The model under review builds one solid part; all positions refer to its coordinate system, in mm. Coordinates: 2 decimals unless noted, no trailing zeros. Loops run counter-clockwise (first coordinate to the right, second up) from the corner with the lowest first, then second, coordinate; pieces in that order, holes last. Notation, with made-up numbers: (63.25, 70) - (79.25, 70) arc R17 ccw to (79.25, 90) - close; hole circle Ø4 at (51, 2.25). An arc over 180 degrees is marked (long way). Answer in a Markdown table with one row per item. Add a question column.
(1) For P1, Ø6, axis at y = -386.5, z = 2, coming from the -X side; P2, Ø3, axis at x = -726, z = 7.5, coming from the +Y side; P3, Ø4, axis at y = -235, z = 6.5, coming from the +X side, all flat-tipped, find the tip position at first contact; note any pin that passes through.
(2) We need section A-A on z = -6.75. Write out the cut boundary in (x, y).
(3) We need section C-C on y = -370. Write out the cut boundary in (x, z), plus the area to 3 significant figures.
(4) For line 1 along Y through (x, z) = (-836.5, -0.25); line 2 along Y through (x, z) = (-935, 2.75); line 3 along X through (y, z) = (-207.5, 0.75), list the stretches that pass through material, from the lowest coordinate up.
(5) We need section B-B on x = -821.5. Write out the cut boundary in (y, z).
from build123d import *

# Parameters (mm, degrees)
SKETCH2_W = 20
SKETCH2_H = 6


with BuildPart() as part:
    # Sweep1: sweep along a path in Sketch1
    with BuildLine(Plane.XY) as sweep1_path:
        Line((-803.471602915, -72.580053696), (-137.514764545, -198.618968438))
        ThreePointArc((-137.514764545, -198.618968438), (-117.217555143, -221.543328014), (-134.339730828, -246.927064367))
        Line((-134.339730828, -246.927064367), (-778.071333179, -459.044821132))
        ThreePointArc((-778.071333179, -459.044821132), (-1040.232770199, -282.208199453), (-803.471602915, -72.580053696))
    # Sketch2 → Sweep1 (sweep)
    with BuildSketch(Plane(origin=(-803.471602915, 0, 0), x_dir=(0, 0, -1), z_dir=(1, 0, 0))):
        with Locations((0, -75.580053696)):
            Rectangle(SKETCH2_W, SKETCH2_H)
    sweep(path=sweep1_path.line)


solid = part.part
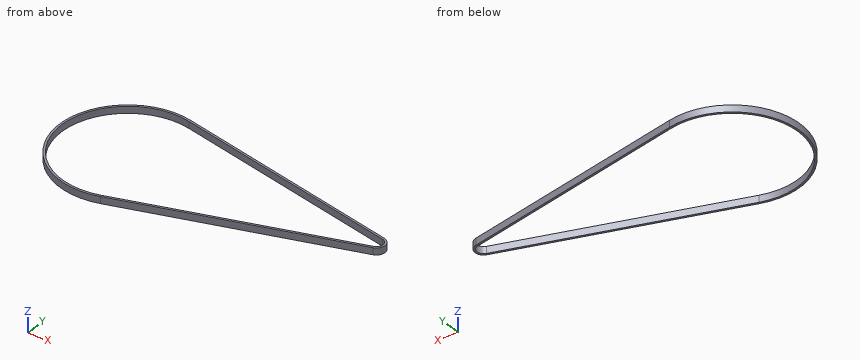
Outcome:
| question | item | result |
|---|---|---|
| 1 | P1 | x = -1004.71 |
| 1 | P2 | y = -86.96 |
| 1 | P3 | x = -119.17 |
| 2 | outline | (-803.47, -72.58) arc R200 ccw (long way) to (-778.07, -459.04) - (-134.34, -246.93) arc R25 ccw to (-137.51, -198.62) - close; hole (-803.47, -78.58) arc R194.11 ccw (long way) to (-780.98, -453.79) - (-137.24, -241.68) arc R19.14 ccw to (-137.51, -204.62) - close |
| 3 | outline | (-1013.34, -10) - (-1006.48, -10) - (-1006.48, 10) - (-1013.34, 10) - close; (-526.68, -10) - (-507.84, -10) - (-507.84, 10) - (-526.68, 10) - close |
| 3 | area | 514 mm² |
| 4 | line 1 | -469.05 to -463.15, -75.03 to -69.13 |
| 4 | line 2 | -445.45 to -438.73, -99.45 to -92.74 |
| 4 | line 3 | -1030.94 to -1024.74, -131.2 to -122.69 |
| 5 | outline | (-468.17, -10) - (-462.25, -10) - (-462.25, 10) - (-468.17, 10) - close; (-75.93, -10) - (-70.01, -10) - (-70.01, 10) - (-75.93, 10) - close |
